from build123d import *

# Parameters (mm, degrees)
SKETCH_2_R          = 10
SKETCH_2_R_2        = 9
CUT_EXTRUDE_1_DEPTH = 2


with BuildPart() as part:
    # 草图1 → 旋转1 (revolve)
    with BuildSketch(Plane.XY):
        Polygon((0, 0), (0, 10), (43, 10), (43, 15), (427, 15), (427, 10), (457, 10), (457, 0), align=None)
    revolve(axis=Axis((457, 0, 0), (-1, 0, 0)))

    # 草图2 → 切除-拉伸1 (cut)
    with BuildSketch(Plane.ZY.offset(-43)):
        with Locations(Location((0, 0, 0), (0, 0, 90))):
            Circle(SKETCH_2_R)
        with Locations(Location((0, 0, 0), (0, 0, 270))):
            Circle(SKETCH_2_R_2, mode=Mode.SUBTRACT)
    extrude(amount=CUT_EXTRUDE_1_DEPTH, mode=Mode.SUBTRACT)


solid = part.part
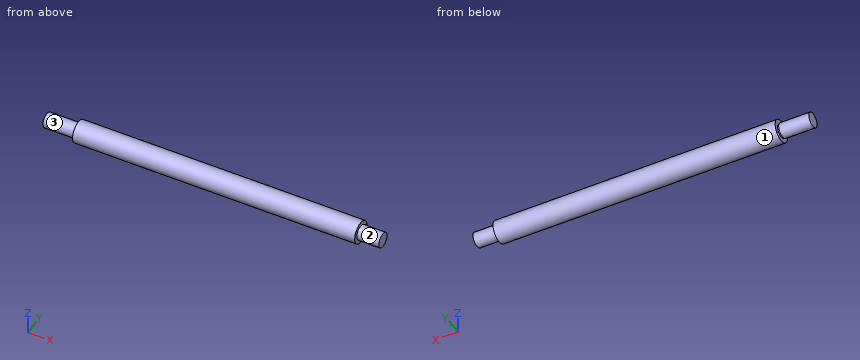
Work out the finished part from the listing and answer in its coordinate system (mm). Face numbers are marked on the shaded views. A direction names the side the tool comes from. Round coordinates to 2 decimals unless told otherwise and drop trailing zeros. Write each loop counter-clockwise with the first axis right and the second up, starting at its lowest first coordinate (ties: lowest second). Pieces come first, ordered by that corner, then holes. Notation, with made-up numbers: (-4.75, 0) -> (19.25, 0) arc R32 cw to (19.25, 26) -> close; hole circle Ø7 at (33, 83.5). An arc over 180 degrees is marked (long way). Write each question's results on one line, items separated by ' | '.
Item 1: Which of the six approach directions +Z, -Z, +X, -X, +Y, -Y give full straight-line access (tool end or side, diameter ignored) to the marked faces 1, 2 and 3?
Result set:
face 1: +X, -X | face 2: +X | face 3: -X
Item 2: Find the intervals of material crossed by line 1 along Z through (x, y) = (184.5, -11.25); line 2 along X through (y, z) = (8.5, -7), in increasing order. Write a range as [from, to].
Result set:
line 1: [-9.92, 9.92] | line 2: [43, 427]
Item 3: A cutting plane is placed at A-A, the plane y = 0. Determine the outline of the cut face in (x, z), plus the area to 3 significant figures.
Result set:
outline: (0, -10) -> (41, -10) -> (41, -9) -> (43, -9) -> (43, -15) -> (427, -15) -> (427, -10) -> (457, -10) -> (457, 10) -> (427, 10) -> (427, 15) -> (43, 15) -> (43, 9) -> (41, 9) -> (41, 10) -> (0, 10) -> close | area: 13,000 mm^2
Item 4: Flat-ended cylindrical pins translate along their axes: P1, Ø6, axis at x = 182, y = 5, coming from the +Z side; P2, Ø1, axis at y = -1, z = 11.5, coming from the -X side; P3, Ø3, axis at x = 291, y = -10, coming from the -Z side. Find the tip coordinate at first contact, or state that the pin passes through.
Result set:
P1: z = 14.87 | P2: x = 43 | P3: z = -12.36
Item 5: A cutting plane is placed at C-C, the plane x = 87. Determine the outline of the cut face in (y, z), plus the area to 3 significant figures.
Result set:
outline: circle Ø30 at (0, 0) | area: 707 mm^2
